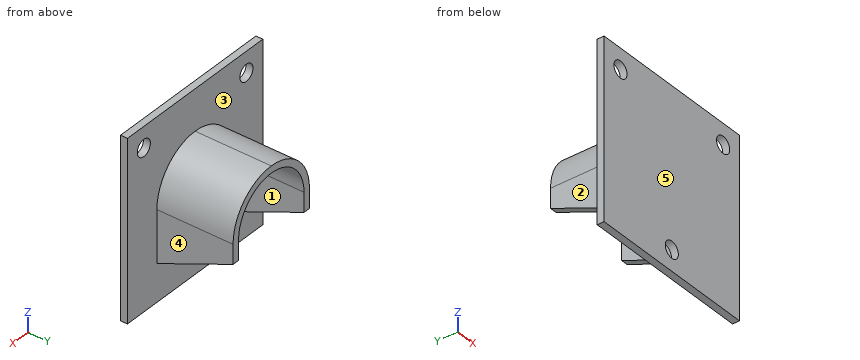
```python
from build123d import *

# Parameters (mm, degrees)
BASE_PLATE_SKETCH_W         = 124
BASE_PLATE_SKETCH_H         = 129
BASE_PLATE_SKETCH_R         = 6
BASE_PLATE_DEPTH            = 5
UPRIGHT_SUPPORT_BLOCK_DEPTH = 35
CRADLE_CUT_SKETCH_W         = 60
CRADLE_CUT_SKETCH_H         = 23.5
CRADLE_CUT_DEPTH            = 55
GUSSET_TRIM_CUT_DEPTH       = 55


with BuildPart() as part:
    # Base Plate Sketch → Base Plate (new body)
    with BuildSketch(Plane(origin=(0, 0, 0), x_dir=(1, 0, 0), z_dir=(0, 1, 0))):
        Rectangle(BASE_PLATE_SKETCH_W, BASE_PLATE_SKETCH_H)
        with Locations(Location((0, 49.5, 0), (0, 0, 270))):
            Circle(BASE_PLATE_SKETCH_R, mode=Mode.SUBTRACT)
        with Locations(Location((47, -49.5, 0), (0, 0, 270))):
            Circle(BASE_PLATE_SKETCH_R, mode=Mode.SUBTRACT)
        with Locations(Location((-47, -49.5, 0), (0, 0, 270))):
            Circle(BASE_PLATE_SKETCH_R, mode=Mode.SUBTRACT)
    extrude(amount=BASE_PLATE_DEPTH)

    # Upright Support Profile Sketch → Upright Support Block (add, symmetric)
    with BuildSketch(Plane(origin=(0, 0, 0), x_dir=(0, 0, -1), z_dir=(1, 0, 0))):
        Polygon((37.5, 5), (14, 60), (-35, 60), (-35, 5), align=None)
    extrude(amount=UPRIGHT_SUPPORT_BLOCK_DEPTH, both=True)

    # Cradle Cut Sketch → Cradle Cut (cut)
    with BuildSketch(Plane(origin=(0, 60, 0), x_dir=(1, 0, 0), z_dir=(0, 1, 0))):
        with Locations((0, 25.75)):
            Rectangle(CRADLE_CUT_SKETCH_W, CRADLE_CUT_SKETCH_H)
        with BuildLine():
            Line((30, 14), (-30, 14))
            Line((-30, 14), (-30, 0))
            ThreePointArc((-30, 0), (0, -30), (30, 0))
            Line((30, 0), (30, 14))
        make_face()
    extrude(amount=-CRADLE_CUT_DEPTH, mode=Mode.SUBTRACT)

    # Gusset Trim Sketch → Gusset Trim Cut (cut)
    with BuildSketch(Plane(origin=(0, 60, 0), x_dir=(1, 0, 0), z_dir=(0, 1, 0))):
        with BuildLine():
            Line((-35, -35), (1.7e-07, -35))
            ThreePointArc((1.7e-07, -35), (-24.748737282, -24.748737402), (-35, 0))
            Line((-35, 0), (-35, -35))
        make_face()
        with BuildLine():
            Line((35, -35), (35, 0))
            ThreePointArc((35, 0), (24.748737402, -24.748737282), (1.7e-07, -35))
            Line((1.7e-07, -35), (35, -35))
        make_face()
    extrude(amount=-GUSSET_TRIM_CUT_DEPTH, mode=Mode.SUBTRACT)


solid = part.part
```
The listing builds one solid part. Answer for the finished solid, in the listing's coordinates (mm). Face numbers are marked on the shaded views. A direction names the side the tool comes from. Give positions to 0.01 mm unless a question says otherwise; leave off trailing zeros. Order: outer loops, then holes, each group sorted by start corner. A loop starts at its lowest first (then second) coordinate and runs counter-clockwise, first axis right, second up.
Item 1: Given pin 1 Ø2 at (x, z) = (9, 23.5) entering from +Y; pin 2 Ø4 at (y, z) = (49.5, 13) entering from -X; pin 3 Ø12 at (y, z) = (8.5, -42) entering from +X; pin 4 Ø19 at (y, z) = (23.5, -19.5) entering from +X, each flat-ended and moving along its own axis, determine where each tip first touches the part or whether it passes through.
From the geometry:
pin 1: stops at y = 5
pin 2: stops at x = -33.23
pin 3: stops at x = 62
pin 4: stops at x = 35
Item 2: The part is cut by section A-A, the plane z = 49.5. Give the vertices of the cut face in (x, y), and give its area (3 significant figures).
From the geometry:
outline: (-62, 0) - (-53, 0) - (-53, 5) - (-62, 5) - close; (-41, 0) - (41, 0) - (41, 5) - (-41, 5) - close; (53, 0) - (62, 0) - (62, 5) - (53, 5) - close
area: 500 mm2
Item 3: For a pull along X with two mould halves and no side action, classify the marked faces 3, 4 and 5 as pulls with the +X half, pulls with the -X half, needs draft (parallel to the pull), parting line crosses it, or undercut.
From the geometry:
face 3: undercut
face 4: pulls with the +X half
face 5: needs draft
Item 4: The part is cut by section D-D, the plane y = 42.5. Give the vertices of the cut face in (x, z), and give its area (3 significant figures).
From the geometry:
outline: (-35, -21.48) - (-30, -21.48) - (-30, 0) arc R30 cw to (30, 0) - (30, -21.48) - (35, -21.48) - (35, 0) arc R35 ccw to (-35, 0) - close
area: 725 mm2
Item 5: Find the intervals of material crossed by probe 1 along X at (y, z) = (2.2, 49.5); probe 2 along X at (y, z) = (3.6, -49.5); probe 3 along X at (y, z) = (33, -25), in increasing order.
From the geometry:
probe 1: x = -62 to -53, -41 to 41, 53 to 62
probe 2: x = -62 to -6, 6 to 62
probe 3: x = -35 to -30, 30 to 35
Item 6: Which of the six approach directions +Z, -Z, +X, -X, +Y, -Y give full straight-line access (tool end or side, diameter ignored) to the marked faces 1 and 2?
From the geometry:
face 1: -Z, +Y
face 2: +Z, -Z, -X, +Y
Item 7: The part is cut by section C-C, the plane z = -49.5. Give the vertices of the cut face in (x, y).
From the geometry:
outline: (-62, 0) - (-6, 0) - (-6, 5) - (-62, 5) - close; (6, 0) - (62, 0) - (62, 5) - (6, 5) - close
Item 8: The part is cut by section B-B, the plane x = -47. Give the vertices of the cut face in (y, z).
From the geometry:
outline: (0, -64.5) - (5, -64.5) - (5, 43.5) - (0, 43.5) - close; (0, 55.5) - (5, 55.5) - (5, 64.5) - (0, 64.5) - close
